from build123d import *

# Parameters (mm, degrees)
EXTRUDE_1_DEPTH    = 10
HOLE_WIZARD_M5_1_D = 4.2


with BuildPart() as part:
    # 草图1 → 凸台-拉伸1 (new, symmetric)
    with BuildSketch(Plane.XY):
        Polygon((0, 0), (-20, 0), (-20, 36), (-12, 36), (-12, 8), (0, 8), align=None)
    extrude(amount=EXTRUDE_1_DEPTH, both=True)

    # M5 螺纹孔1 (through all)
    with Locations(Plane(origin=(-20, 30, 0), x_dir=(0, 0, -1), z_dir=(-1, 0, 0))):
        with Locations((0, 0)):
            Hole(HOLE_WIZARD_M5_1_D / 2)


solid = part.part
Input: part model. Units: mm. Frame: model coordinates. A direction names the side the tool comes from. Coordinates: 2 decimals unless noted, no trailing zeros. Order: outer loops, then holes, each group sorted by start corner. A loop starts at its lowest first (then second) coordinate and runs counter-clockwise, first axis right, second up. Notation, with made-up numbers: M -3,56 L 56,56 A30 ccw 56,88 Z; hole C -12,-37.5 d8. An arc over 180 degrees is marked long. Write item = value, one per line. Start each with the question number.
(1) Section B-B on y = 30. Output: boundary loops of the cut face in (x, z).
(2) Reachability of faces 1 (the flat face through (-20, 18, 0)), 2 (the flat face through (-12, 22, 0)) from +Z, -Z, +X, -X, +Y, -Y: full face, straight path, thin tool, end or side. Return the list, or none.
(3) First-contact query: P1, Ø12, axis at x = -14, z = 0, coming from the -Y side; P2, Ø6, axis at y = 17.5, z = 1.5, coming from the +X side; P3, Ø6, axis at x = -3.5, z = 2.5, coming from the +Y side. Flat tips, straight axial feed; report the tip coordinate or a pass-through.
(4) Pull-direction query (Y, two-part tool) for faces 3 (the flat face through (-10, 0, 0)), 4 (the cylindrical face through (-15.944, 31.863, 0.969)), 5 (the flat face through (0, 4, 0)); classes: released by +Y, released by -Y, zero draft, split by the parting line, or undercut.
(5) Section C-C on x = -2. Output: boundary loops of the cut face in (y, z).
(6) Section A-A on z = 0. Output: boundary loops of the cut face in (x, y), and give its area (3 significant figures).
(7) Line query: line 1 along Y through (x, z) = (-15, 0); line 2 along Z through (x, y) = (-14.25, 30); line 3 along X through (y, z) = (11, -2.5). Output: solid intervals per line, ascending. Write a range as [from, to].
(8) Section D-D on z = 7.75. Output: boundary loops of the cut face in (x, y), and give its area (3 significant figures).
Result set:
q1.outline = M -20,-10 L -12,-10 L -12,-2.1 L -20,-2.1 Z; M -20,2.1 L -12,2.1 L -12,10 L -20,10 Z
q2.face_1 = +Z, -Z, -X, +Y, -Y
q2.face_2 = +Z, -Z, +X, +Y
q3.P1 = 0
q3.P2 = -12
q3.P3 = 8
q4.face_3 = released by -Y
q4.face_4 = undercut
q4.face_5 = zero draft
q5.outline = M 0,-10 L 8,-10 L 8,10 L 0,10 Z
q6.outline = M -20,0 L 0,0 L 0,8 L -12,8 L -12,27.9 L -20,27.9 Z; M -20,32.1 L -12,32.1 L -12,36 L -20,36 Z
q6.area = 350 mm²
q7.line_1 = [0, 27.9], [32.1, 36]
q7.line_2 = [-10, -2.1], [2.1, 10]
q7.line_3 = [-20, -12]
q8.outline = M -20,0 L 0,0 L 0,8 L -12,8 L -12,36 L -20,36 Z
q8.area = 384 mm²
